```python
from build123d import *

# Parameters (mm, degrees)
CIRPATTERN1_COUNT = 4


with BuildPart() as part:
    # Sketch1 → Revolve1 (revolve)
    with BuildSketch(Plane.XY, mode=Mode.PRIVATE) as revolve1_sk:
        Polygon((0, 16), (0, 35), (8, 35), (8, 23.5), (15, 23.5), (15, 26), (50, 26), (50, 16), align=None)
    revolve(revolve1_sk.sketch.rotate(Axis((0, 0, 0), (1, 0, 0)), 90), axis=Axis((0, 0, 0), (1, 0, 0)))

    # Sketch3 → Ø10.0 (10) Diameter Hole1 (revolve, cut)
    with BuildSketch(Plane.ZX.offset(25)):
        Polygon((0, 0), (0, 7.004303095), (5, 4), (5, 0), align=None)
    f_10_0_10_diameter_hole1 = revolve(axis=Axis((-6.35, 25, 0), (1, 0, 0)), mode=Mode.SUBTRACT)

    # CirPattern1: Ø10.0 (10) Diameter Hole1 ×4 about axis
    cirpattern1_axis = Axis((0, 0, 0), (1, 0, 0))
    for i in range(1, CIRPATTERN1_COUNT):
        add(f_10_0_10_diameter_hole1.rotate(cirpattern1_axis, i * 360 / CIRPATTERN1_COUNT), mode=Mode.SUBTRACT)


solid = part.part
```
Input: part model. Units: mm. Frame: model coordinates. A direction names the side the tool comes from. Give positions to 0.01 mm unless a question says otherwise; leave off trailing zeros. Loops run counter-clockwise (first coordinate to the right, second up) from the corner with the lowest first, then second, coordinate; pieces in that order, holes last. Notation, with made-up numbers: (28, 29) -> (44, 29) arc R16 ccw to (44, 36) -> close; hole circle Ø10 at (70.5, 67). An arc over 180 degrees is marked (long way). Use a Markdown table: item, result.
Q1. First-contact query: P1, Ø4, axis at y = -21, z = -23.5, coming from the +X side; P2, Ø2, axis at x = 9.5, z = 4, coming from the +Y side; P3, Ø1.5, axis at x = 23, z = -11.5, coming from the -Y side. Flat tips, straight axial feed; report the tip coordinate or a pass-through.
Entries:
| item | result |
|---|---|
| P1 | stops at x = 8 |
| P2 | stops at y = 23.31 |
| P3 | stops at y = -23.67 |
Q2. Access query for faces 1 (the flat face through (50, -12, 11)), 2 (the cylindrical face through (1.97, 29.88, -1.08)), 3 (the flat face through (15, 23, 6)). Directions: +Z, -Z, +X, -X, +Y, -Y. A direction counts if a zero-diameter tool reaches every point of the face in a straight line with its end or side. Return the directions, or none.
Entries:
| item | result |
|---|---|
| face 1 | +Z, -Z, +X, +Y, -Y |
| face 2 | -X |
| face 3 | none |
Q3. Section query A-A, the plane z = -14. Return the cut outline in (x, y).
Entries:
| item | result |
|---|---|
| outline | (0, -32.08) -> (8, -32.08) -> (8, -18.87) -> (15, -18.87) -> (15, -21.91) -> (50, -21.91) -> (50, -7.75) -> (0, -7.75) -> close; (0, 7.75) -> (50, 7.75) -> (50, 21.91) -> (15, 21.91) -> (15, 18.87) -> (8, 18.87) -> (8, 32.08) -> (0, 32.08) -> close |
Q4. Section query B-B, the plane x = 28. Return the cut outline in (y, z).
Entries:
| item | result |
|---|---|
| outline | circle Ø52 at (0, 0); hole circle Ø32 at (0, 0) |
Q5. Pull-direction query (Z, two-part tool) for faces 4 (the cylindrical face through (32.745, 15.821, -20.633)), 5 (the conical face through (6.483, 24.268, 0.467)), 6 (the cylindrical face through (1.97, -1.08, -29.88)), 7 (the flat face through (8, 23, 7)); classes: pulls with the +Z half, pulls with the -Z half, needs draft (parallel to the pull), parting line crosses it, or undercut.
Entries:
| item | result |
|---|---|
| face 4 | parting line crosses it |
| face 5 | undercut |
| face 6 | undercut |
| face 7 | needs draft |
Q6. Section query C-C, the plane z = 6. Return the cut outline in (x, y).
Entries:
| item | result |
|---|---|
| outline | (0, -34.48) -> (8, -34.48) -> (8, -22.72) -> (15, -22.72) -> (15, -25.3) -> (50, -25.3) -> (50, -14.83) -> (0, -14.83) -> close; (0, 14.83) -> (50, 14.83) -> (50, 25.3) -> (15, 25.3) -> (15, 22.72) -> (8, 22.72) -> (8, 34.48) -> (0, 34.48) -> close |
Q7. Ray query, probe 1 along Y at (x, z) = (33, 0); probe 2 along X at (y, z) = (12.5, -21); probe 3 along Z at (x, y) = (19, -20.5). Return the intervals inside material, ascending. Write a range as from..to.
Entries:
| item | result |
|---|---|
| probe 1 | y = -26..-16, 16..26 |
| probe 2 | x = 0..8, 15..50 |
| probe 3 | z = -15.99..15.99 |
